from build123d import *

# Parameters (mm, degrees)
SADDLE_BODY_DEPTH     = 25
EDGE_FILLETS_R2_R     = 2
CORNER_FILLETS_R7_R   = 7
FLANGE_HOLES_SKETCH_R = 4
FLANGE_HOLES_DEPTH    = 50
U_SLOT_CUT_DEPTH      = 20


with BuildPart() as part:
    # Saddle Profile Sketch → Saddle Body (new, symmetric)
    with BuildSketch(Plane.XY):
        with BuildLine():
            Line((-58, 0), (-23, 0))
            ThreePointArc((-23, 0), (0, 23), (23, 0))
            Line((23, 0), (57, 0))
            Line((57, 0), (57, 42))
            Line((57, 42), (48, 42))
            Line((48, 42), (48, 9))
            Line((48, 9), (30.708305066, 9))
            ThreePointArc((30.708305066, 9), (0, 32), (-30.708305066, 9))
            Line((-30.708305066, 9), (-58, 9))
            Line((-58, 9), (-58, 0))
        make_face()
    extrude(amount=SADDLE_BODY_DEPTH, both=True)

    # Edge Fillets R2
    edge_fillets_r2_edges = [part.edges().sort_by_distance(p)[0] for p in [
        (-30.708305066, 9, 0),
        (30.708305066, 9, 0),
        (48, 9, 0),
    ]]
    fillet(edge_fillets_r2_edges, radius=EDGE_FILLETS_R2_R)

    # Corner Fillets R7
    corner_fillets_r7_edges = [part.edges().sort_by_distance(p)[0] for p in [
        (-58, 4.5, -25),
        (52.5, 42, -25),
        (52.5, 42, 25),
        (-58, 4.5, 25),
    ]]
    fillet(corner_fillets_r7_edges, radius=CORNER_FILLETS_R7_R)

    # Flange Holes Sketch → Flange Holes (cut)
    with BuildSketch(Plane(origin=(0, 9, 0), x_dir=(1, 0, 0), z_dir=(0, 1, 0))):
        with Locations(Location((-51, 18, 0), (0, 0, 180))):
            Circle(FLANGE_HOLES_SKETCH_R)
        with Locations(Location((-51, -18, 0), (0, 0, 180))):
            Circle(FLANGE_HOLES_SKETCH_R)
    extrude(amount=-FLANGE_HOLES_DEPTH, mode=Mode.SUBTRACT)

    # U-Slot Sketch → U-Slot Cut (cut)
    with BuildSketch(Plane(origin=(57, 0, 0), x_dir=(0, 0, -1), z_dir=(1, 0, 0))):
        with BuildLine():
            Line((-6, 24), (-6, 44.935144294))
            ThreePointArc((-6, 44.935144294), (0, 50.935144294), (6, 44.935144294))
            Line((6, 44.935144294), (6, 24))
            ThreePointArc((6, 24), (0, 18), (-6, 24))
        make_face()
    extrude(amount=-U_SLOT_CUT_DEPTH, mode=Mode.SUBTRACT)


solid = part.part
Read the model definition and answer for the solid it produces. Units are mm, in the model's axes. A direction names the side the tool comes from. Coordinates: 2 decimals unless noted, no trailing zeros. Loops run counter-clockwise (first coordinate to the right, second up) from the corner with the lowest first, then second, coordinate; pieces in that order, holes last.
Q1. Each of these flat-tipped pins is pushed along its axis until it touches: pin 1 Ø11 at (x, z) = (38, -8) entering from +Y; pin 2 Ø12 at (x, y) = (-23, 33.5) entering from +Z; pin 3 Ø4 at (x, z) = (-7, 19) entering from +Y; pin 4 Ø2 at (x, z) = (-5.5, -15) entering from -Y. Where does it stop, or does it pass through?
Q2. The part is cut by section D-D on x = 0. Write down the section's boundary in (y, z), and give its area (3 significant figures).
Q3. Which of the six approach directions +Z, -Z, +X, -X, +Y, -Y give full straight-line access (tool end or side, diameter ignored) to faces 1 (the face through (-45, 9, 0)), 2 (the face through (52.4, 39.9, -23)), 3 (the face through (39, 9, 0)), 4 (the face through (53, 33, 6))?
Q4. Consider probe 1 along Z at (x, y) = (-51, 3.25); probe 2 along X at (y, z) = (10.5, -19); probe 3 along Y at (x, z) = (-1, -20). Determine where each line is inside the solid, lowest interval first.
Q5. The part is cut by section A-A on y = 4.5. Write down the section's boundary in (x, z), and give its area (3 significant figures).
Q6. The part is cut by section C-C on z = 0. Write down the section's boundary in (x, y), and give its area (3 significant figures).
Q7. The part is cut by section B-B on z = -15.5. Write down the section's boundary in (x, y).
Q8. The mould has two halves that part along Z. Classify faces 5 (the face through (53, 42, 12)), 6 (the face through (-55.9, 4.4, -23)), 7 (the face through (-48.05, 4.56, 20.7)): +Z half, -Z half, draft (parallel to the pull), parting line (faces both ways), or undercut.
Results below:
1. pin 1: stops at y = 9
1. pin 2: passes through
1. pin 3: stops at y = 31.61
1. pin 4: stops at y = 22.06
2. outline: (23, -25) - (32, -25) - (32, 25) - (23, 25) - close
2. area: 450 mm2
3. face 1: +Z, -Z, -X, +Y
3. face 2: -Z, +X, -X, +Y
3. face 3: +Z, -Z, +Y
3. face 4: +X, +Y
4. probe 1: z = -25 to -22, -14 to 14, 22 to 25
4. probe 2: x = -30.23 to -20.46, 20.46 to 30.23, 47.94 to 57
4. probe 3: y = 22.98 to 31.98
5. outline: (-58, -18) arc R7 ccw to (-51, -25) - (-22.56, -25) - (-22.56, 25) - (-51, 25) arc R7 ccw to (-58, 18) - close; (22.56, -25) - (57, -25) - (57, 25) - (22.56, 25) - close; hole circle Ø8 at (-51, -18); hole circle Ø8 at (-51, 18)
5. area: 3,370 mm2
6. outline: (-58, 0) - (-23, 0) arc R23 cw to (23, 0) - (57, 0) - (57, 18) - (48, 18) - (48, 11) arc R2 cw to (46, 9) - (32.17, 9) arc R2 cw to (30.28, 10.35) arc R32 ccw to (-30.28, 10.35) arc R2 cw to (-32.17, 9) - (-58, 9) - close
6. area: 1,330 mm2
7. outline: (-58, 0) - (-54.12, 0) - (-54.12, 9) - (-58, 9) - close; (-47.88, 0) - (-23, 0) arc R23 cw to (23, 0) - (57, 0) - (57, 42) - (48, 42) - (48, 11) arc R2 cw to (46, 9) - (32.17, 9) arc R2 cw to (30.28, 10.35) arc R32 ccw to (-30.28, 10.35) arc R2 cw to (-32.17, 9) - (-47.88, 9) - close
8. face 5: draft
8. face 6: -Z half
8. face 7: undercut
